from build123d import *

# Parameters (mm, degrees)
EXTRUDE_1_DEPTH = 1185


with BuildPart() as part:
    # 草图1 → 拉伸1 (new body)
    with BuildSketch(Plane.XY):
        with BuildLine():
            Line((0, 0), (0, 40))
            Line((0, 40), (3.99, 40))
            ThreePointArc((3.99, 40), (3.997071068, 39.997071068), (4, 39.99))
            Line((4, 39.99), (4, 9))
            ThreePointArc((4, 9), (5.464466094, 5.464466094), (9, 4))
            Line((9, 4), (39.99, 4))
            ThreePointArc((39.99, 4), (39.997071068, 3.997071068), (40, 3.99))
            Line((40, 3.99), (40, 0))
            Line((40, 0), (0, 0))
        make_face()
    extrude(amount=EXTRUDE_1_DEPTH)


solid = part.part
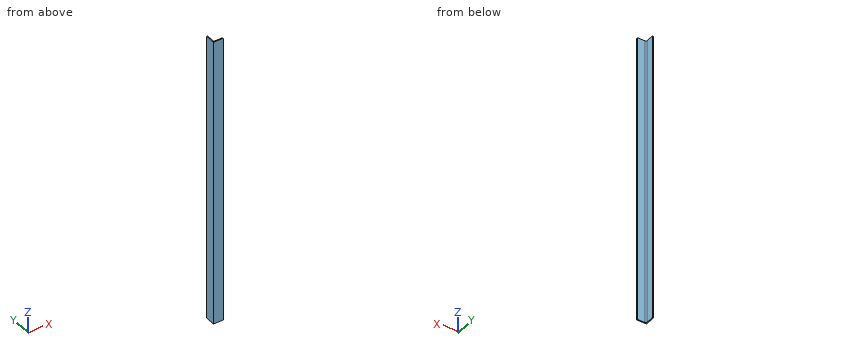
Work out the finished part from the listing and answer in its coordinate system (mm). Give positions to 0.01 mm unless a question says otherwise; leave off trailing zeros. Write each loop counter-clockwise with the first axis right and the second up, starting at its lowest first coordinate (ties: lowest second). Pieces come first, ordered by that corner, then holes. Notation, with made-up numbers: (73.5, 31.25) - (120.5, 31.25) arc R28 ccw to (120.5, 61.25) - close; hole circle Ø7 at (-29, -17). An arc over 180 degrees is marked (long way). One line per item, written item: value. Start each with the question number.
1. Consider probe 1 along X at (y, z) = (16, 734); probe 2 along Y at (x, z) = (5.5, 1076.5). Determine where each line is inside the solid, lowest interval first.
2. Given pin 1 (9.5 mm diameter, centred on y = 27.5, z = 578, fed in from +X); pin 2 (15.5 mm diameter, centred on x = 21, z = 589, fed in from +Y); pin 3 (5 mm diameter, centred on y = 28.5, z = 602, fed in from -X), each flat-ended and moving along its own axis, determine where each tip first touches the part or whether it passes through.
3. Find section B-B (y = 15.5). Write down the section's boundary in (x, z).
Geometry results:
1. probe 1: 0 to 4
1. probe 2: 0 to 5.43
2. pin 1: x = 4
2. pin 2: y = 4
2. pin 3: x = 0
3. outline: (0, 0) - (4, 0) - (4, 1185) - (0, 1185) - close
